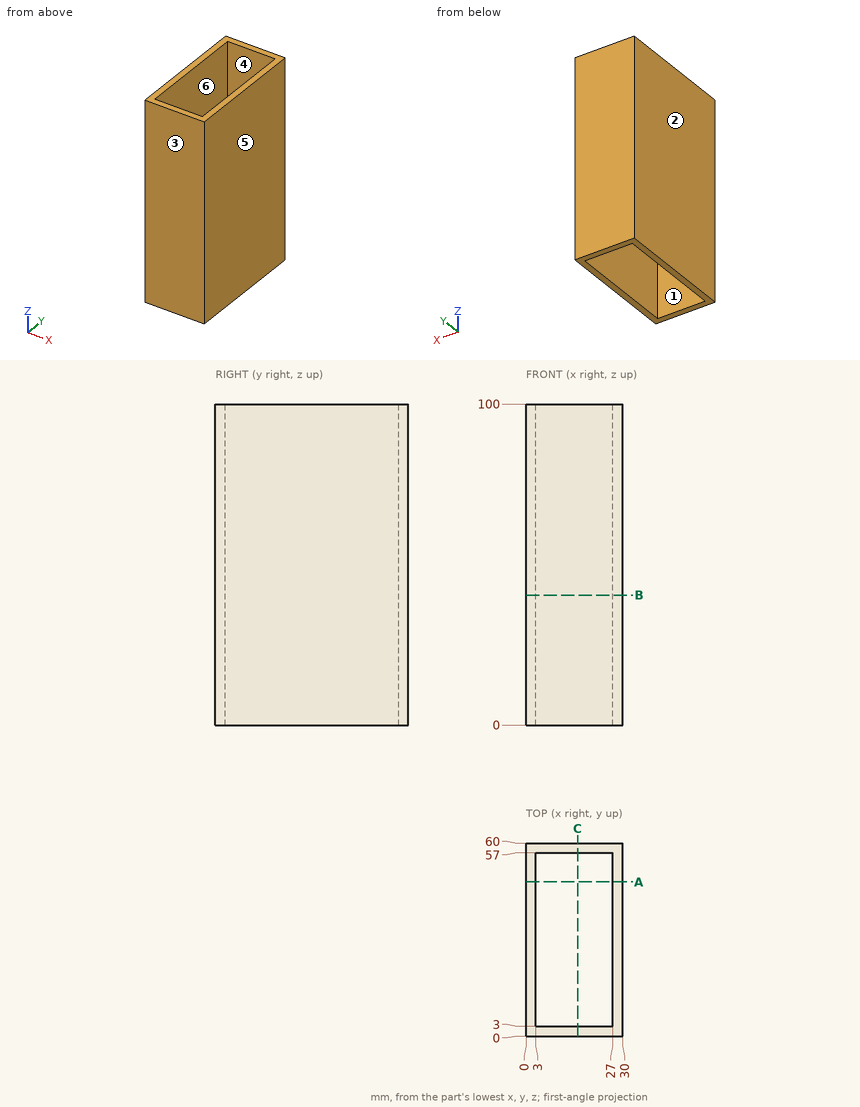
Can you work these out from the drawing? Everything is in mm from the part's minimum corner. A direction names the side the tool comes from. Give positions to 0.01 mm unless a question says otherwise; leave off trailing zeros. Order: outer loops, then holes, each group sorted by start corner. A loop starts at its lowest first (then second) coordinate and runs counter-clockwise, first axis right, second up. Notation, with made-up numbers: (5, -0.5) -> (46, -0.5) arc R29 cw to (46, 26.5) -> close; hole circle Ø4 at (35.5, -11). An arc over 180 degrees is marked (long way). Return JSON: item names as keys, results as strings.
1. Imagine slicing it at B-B on z = 40.5. List the corners of the cut face in (x, y) for me, then the cut area to 3 significant figures.
Answer list:
{"outline": "(0, 0) -> (30, 0) -> (30, 60) -> (0, 60) -> close; hole (3, 3) -> (27, 3) -> (27, 57) -> (3, 57) -> close", "area": "504 mm2"}
2. Imagine slicing it at A-A on y = 48. List the corners of the cut face in (x, z) for me, then the cut area to 3 significant figures.
Answer list:
{"outline": "(0, 0) -> (3, 0) -> (3, 100) -> (0, 100) -> close; (27, 0) -> (30, 0) -> (30, 100) -> (27, 100) -> close", "area": "600 mm2"}
3. Imagine slicing it at C-C on x = 16. List the corners of the cut face in (y, z) for me.
Answer list:
{"outline": "(0, 0) -> (3, 0) -> (3, 100) -> (0, 100) -> close; (57, 0) -> (60, 0) -> (60, 100) -> (57, 100) -> close"}
4. On a 3-axis mill with a long thin cutter (end or side, diameter ignored), from which of +Z, -Z, +X, -X, +Y, -Y can I reach the whole of each face in a straight line? I mean the marked faces 5 and 6. Say none if no direction works.
Answer list:
{"face 5": "+Z, -Z, +X, +Y, -Y", "face 6": "+Z, -Z"}
5. Thinking about a two-plate mould opening in X: for the marked faces 1, 2, 3 and 4, which applies, pulls with the +X half, pulls with the -X half, needs draft (parallel to the pull), parting line crosses it, or undercut?
Answer list:
{"face 1": "undercut", "face 2": "pulls with the -X half", "face 3": "needs draft", "face 4": "undercut"}
6. I need wall thicknesses on line 1 (X direction, y = 12, z = 75.5); line 2 (Y direction, x = 20.75, z = 90). Which ranges of each line are inside material? Lowest first, please. Write a range as from..to.
Answer list:
{"line 1": "x = 0..3, 27..30", "line 2": "y = 0..3, 57..60"}
